The figure shows three views and two pictorial views of one solid part (mm, origin at its lowest corner). Answer the questions. Coordinates: 2 decimals unless noted, no trailing zeros. Order: outer loops, then holes, each group sorted by start corner. A loop starts at its lowest first (then second) coordinate and runs counter-clockwise, first axis right, second up.
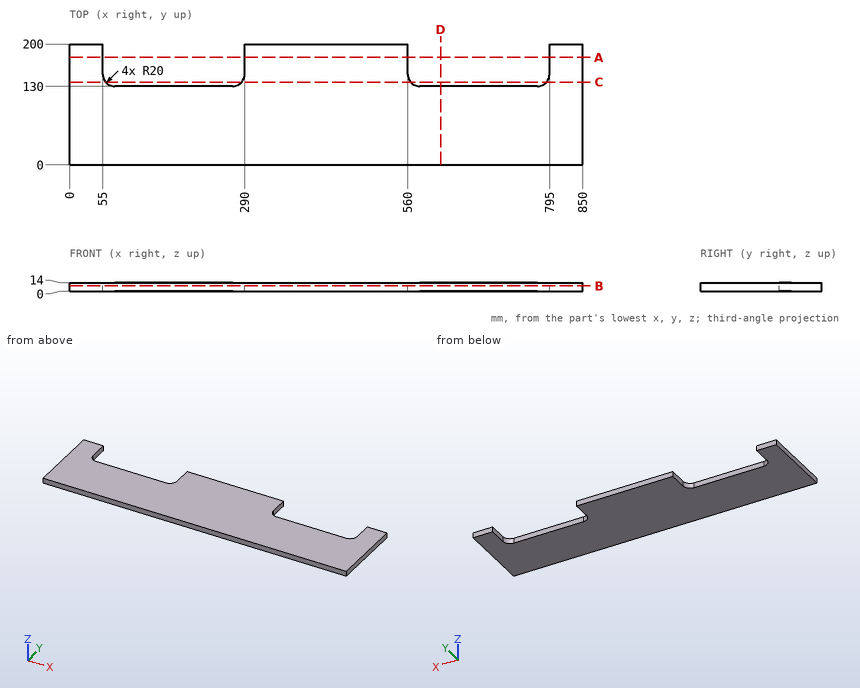
1) A cutting plane is placed at B-B, the plane z = 9. Write down the section's boundary in (x, y).
2) A cutting plane is placed at A-A, the plane y = 178. Write down the section's boundary in (x, z).
3) A cutting plane is placed at D-D, the plane x = 614.5. Write down the section's boundary in (y, z), plus the area to 3 significant figures.
4) This flat-tipped pin is pushed along its axis until it touches: P1, Ø1.5, axis at x = 755, z = 7, coming from the +Y side. Where does it stop, or does it pass through?
5) Straight lines are drawn through the part: probe 1 along X at (y, z) = (184.5, 6.25); probe 2 along Y at (x, z) = (740.5, 2); probe 3 along X at (y, z) = (144, 3.75). For each, find the intervals that lie inside material, in ascending order.
6) A cutting plane is placed at C-C, the plane y = 137. Write down the section's boundary in (x, z).
Working result:
1. outline: (0, 0) - (850, 0) - (850, 200) - (795, 200) - (795, 150) arc R20 cw to (775, 130) - (580, 130) arc R20 cw to (560, 150) - (560, 200) - (290, 200) - (290, 150) arc R20 cw to (270, 130) - (75, 130) arc R20 cw to (55, 150) - (55, 200) - (0, 200) - close
2. outline: (0, 0) - (55, 0) - (55, 14) - (0, 14) - close; (290, 0) - (560, 0) - (560, 14) - (290, 14) - close; (795, 0) - (850, 0) - (850, 14) - (795, 14) - close
3. outline: (0, 0) - (130, 0) - (130, 14) - (0, 14) - close
3. area: 1,820 mm2
4. P1: stops at y = 130
5. probe 1: x = 0 to 55, 290 to 560, 795 to 850
5. probe 2: y = 0 to 130
5. probe 3: x = 0 to 55.92, 289.08 to 560.92, 794.08 to 850
6. outline: (0, 0) - (59.8, 0) - (59.8, 14) - (0, 14) - close; (285.2, 0) - (564.8, 0) - (564.8, 14) - (285.2, 14) - close; (790.2, 0) - (850, 0) - (850, 14) - (790.2, 14) - close
